from build123d import *

# Parameters (mm, degrees)
CUT_EXTRUDE3_DEPTH    = 10
CHAMFER2_SIZE         = 0.5
M3_TAPPED_HOLE1_D     = 2.5
M3_TAPPED_HOLE1_DEPTH = 8.5
M3_TAPPED_HOLE1_TIP   = 0.751075774
M4_TAPPED_HOLE1_D     = 3.3
M4_TAPPED_HOLE1_DEPTH = 11.5
M4_TAPPED_HOLE1_TIP   = 0.991420021
SKETCH16_R            = 1.5
CUT_EXTRUDE4_DEPTH    = 26.5


with BuildPart() as part:
    # Sketch1 → Revolve1 (revolve)
    with BuildSketch(Plane.XY, mode=Mode.PRIVATE) as revolve1_sk:
        Polygon((10, 51), (10, 4), (25, 4), (25, 0), (6, 0), (6, 51), align=None)
    revolve(revolve1_sk.sketch.rotate(Axis((0, 57.582524272, 0), (0, -1, 0)), 90), axis=Axis((0, 57.582524272, 0), (0, -1, 0)))

    # Sketch9 → Cut-Extrude3 (cut)
    with BuildSketch(Plane(origin=(0, 4, 0), x_dir=(1, 0, 0), z_dir=(0, 1, 0))):
        with BuildLine():
            Line((-26.167728216, -12.5), (26.167728216, -12.5))
            ThreePointArc((26.167728216, -12.5), (0, -29), (-26.167728216, -12.5))
        make_face()
        with BuildLine():
            Line((-26.167728216, 12.5), (26.167728216, 12.5))
            ThreePointArc((26.167728216, 12.5), (0, 29), (-26.167728216, 12.5))
        make_face()
    extrude(amount=-CUT_EXTRUDE3_DEPTH, mode=Mode.SUBTRACT)

    # Chamfer2
    chamfer2_edges = [part.edges().sort_by_distance(p)[0] for p in [
        (-25, 4, 0),
        (0, 4, -12.5),
        (25, 4, 0),
        (0, 4, 12.5),
        (0, 51, -6),
        (0, 51, -10),
    ]]
    chamfer(chamfer2_edges, length=CHAMFER2_SIZE)

    # M3 Tapped Hole1
    with Locations(Plane(origin=(0, 22, 10), x_dir=(1, 0, 0), z_dir=(0, 0, 1))):
        with Locations((0, 0), (0, 24)):
            Hole(M3_TAPPED_HOLE1_D / 2, depth=M3_TAPPED_HOLE1_DEPTH)
            with Locations((0, 0, -(M3_TAPPED_HOLE1_DEPTH + M3_TAPPED_HOLE1_TIP / 2))):  # 118° drill point
                Cone(0, M3_TAPPED_HOLE1_D / 2, M3_TAPPED_HOLE1_TIP, mode=Mode.SUBTRACT)

    # M4 Tapped Hole1
    with Locations(Plane(origin=(-20, 0, 0), x_dir=(0, 0, -1), z_dir=(0, -1, 0))):
        with Locations((0, 0), (0, 40)):
            Hole(M4_TAPPED_HOLE1_D / 2, depth=M4_TAPPED_HOLE1_DEPTH)
            with Locations((0, 0, -(M4_TAPPED_HOLE1_DEPTH + M4_TAPPED_HOLE1_TIP / 2))):  # 118° drill point
                Cone(0, M4_TAPPED_HOLE1_D / 2, M4_TAPPED_HOLE1_TIP, mode=Mode.SUBTRACT)

    # Sketch16 → Cut-Extrude4 (cut, symmetric)
    with BuildSketch(Plane(origin=(0, 0, 0), x_dir=(0, 0, -1), z_dir=(1, 0, 0))):
        with Locations((0, 14)):
            Circle(SKETCH16_R)
    extrude(amount=CUT_EXTRUDE4_DEPTH, both=True, mode=Mode.SUBTRACT)


solid = part.part
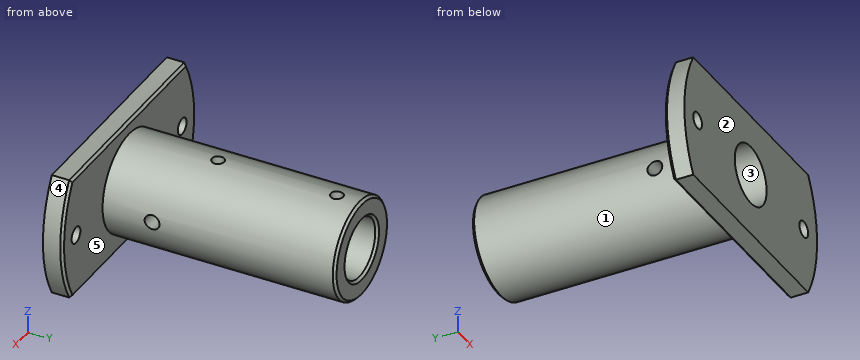
Geometry: final body of the model. Coordinates: model frame, mm. Face numbers are marked on the shaded views. A direction names the side the tool comes from. Round coordinates to 2 decimals unless told otherwise and drop trailing zeros. Loops run counter-clockwise (first coordinate to the right, second up) from the corner with the lowest first, then second, coordinate; pieces in that order, holes last.
Q1. Section D-D on x = 20. Return loops of the section in (y, z), plus the area to 4 significant figures.
Q2. Material intervals for L1, parallel to X at y = 20, z = 0.25; L2, parallel to Y at x = 8.3, z = 0; L3, parallel to Y at x = -13, z = 7.75, sorted ascending.
Q3. Access query for the marked faces 1 and 2. Directions: +Z, -Z, +X, -X, +Y, -Y. A direction counts if a zero-diameter tool reaches every point of the face in a straight line with its end or side. Return the directions, or none.
Q4. Section B-B on z = 0. State how many separate pieces and enclosed holes the cut face has, plus the area to 3 significant figures.
Q5. Section A-A on x = 0. Return loops of the section in (y, z).
Q6. Section C-C on y = 14. Return loops of the section in (x, z), plus the area to 3 significant figures.
Q7. Pull-direction query (X, two-part tool) for the marked faces 3, 4 and 5; classes: released by +X, released by -X, zero draft, split by the parting line, or undercut.
Q8. Pin query (flat end, axial travel): P1, Ø6, axis at x = 18.5, z = -3.5, coming from the -Y side; P2, Ø4.5, axis at x = -20, z = 0, coming from the +Y side; P3, Ø2.5, axis at x = 20, z = 0, coming from the +Y side; P4, Ø2, axis at y = 41.5, z = 6.5, coming from the -X side. Return the tip coordinate at first contact, or that it passes through.
Evaluation:
1. outline: (0, -12.5) - (3.5, -12.5) - (4, -12) - (4, -1.65) - (0, -1.65) - close; (0, 1.65) - (4, 1.65) - (4, 12) - (3.5, 12.5) - (0, 12.5) - close
1. area: 86.55 mm2
2. L1: x = -10 to -5.99, 5.99 to 10
2. L2: y = 0 to 12.5, 15.5 to 51
2. L3: y = 0 to 4
3. face 1: +Y
3. face 2: +Z, -Z, +X, -X, -Y
4. separate pieces: 6
4. enclosed holes: 0
4. area: 477 mm2
5. outline: (0, -12.5) - (3.5, -12.5) - (4, -12) - (4, -10) - (50.5, -10) - (51, -9.5) - (51, -6.5) - (50.5, -6) - (0, -6) - close; (0, 6) - (20.75, 6) - (20.75, 10) - (4, 10) - (4, 12) - (3.5, 12.5) - (0, 12.5) - close; (23.25, 6) - (44.75, 6) - (44.75, 10) - (23.25, 10) - close; (47.25, 6) - (50.5, 6) - (51, 6.5) - (51, 9.5) - (50.5, 10) - (47.25, 10) - close
6. outline: (-9.89, -1.5) arc R10 ccw to (9.89, -1.5) - (5.81, -1.5) arc R6 cw to (-5.81, -1.5) - close; (-9.89, 1.5) - (-5.81, 1.5) arc R6 cw to (5.81, 1.5) - (9.89, 1.5) arc R10 ccw to start
6. area: 177 mm2
7. face 3: undercut
7. face 4: released by +X
7. face 5: zero draft
8. P1: stops at y = 0
8. P2: stops at y = 4
8. P3: passes through
8. P4: stops at x = -8.35
